Check sheet for the modelled part. Datum: model origin and axes. Units: mm. Face numbers are marked on the shaded views. A direction names the side the tool comes from. Coordinates: 2 decimals unless noted, no trailing zeros. Loops run counter-clockwise (first coordinate to the right, second up) from the corner with the lowest first, then second, coordinate; pieces in that order, holes last.
```python
from build123d import *

# Parameters (mm, degrees)
SKETCH_1_R              = 22.5
EXTRUDE_1_DEPTH         = 705
SKETCH_2_R              = 20.5
EXTRUDE_2_DEPTH         = 39
SKETCH_3_R              = 20
EXTRUDE_3_DEPTH         = 37
SKETCH_4_R              = 19.5
EXTRUDE_4_DEPTH         = 60
SKETCH_5_R              = 17.5
EXTRUDE_5_DEPTH         = 18
EXTRUDE_START           = 39
SKETCH_6_R              = 20.5
EXTRUDE_6_DEPTH         = 39
EXTRUDE_START_2         = 37
SKETCH_7_R              = 20
EXTRUDE_7_DEPTH         = 37
CHAMFER_1_SIZE          = 1
CUT_EXTRUDE_1_DEPTH     = 5.9
CUT_EXTRUDE_2_DEPTH     = 5.73
HOLE_WIZARD_M10_1_D     = 8.5
HOLE_WIZARD_M10_1_DEPTH = 15
HOLE_WIZARD_M10_1_TIP   = 2.553657631


with BuildPart() as part:
    # 草图1 → 凸台-拉伸1 (new body)
    with BuildSketch(Plane(origin=(0, 0, 0), x_dir=(0, 0, -1), z_dir=(1, 0, 0))):
        Circle(SKETCH_1_R)
    extrude(amount=EXTRUDE_1_DEPTH)

    # 草图2 → 凸台-拉伸2 (add)
    with BuildSketch(Plane(origin=(705, 0, 0), x_dir=(0, 0, -1), z_dir=(1, 0, 0))):
        Circle(SKETCH_2_R)
    extrude(amount=EXTRUDE_2_DEPTH)

    # 草图3 → 凸台-拉伸3 (add)
    with BuildSketch(Plane(origin=(744, 0, 0), x_dir=(0, 0, -1), z_dir=(1, 0, 0))):
        Circle(SKETCH_3_R)
    extrude(amount=EXTRUDE_3_DEPTH)

    # 草图4 → 凸台-拉伸4 (add)
    with BuildSketch(Plane(origin=(781, 0, 0), x_dir=(0, 0, -1), z_dir=(1, 0, 0))):
        Circle(SKETCH_4_R)
    extrude(amount=EXTRUDE_4_DEPTH)

    # 草图5 → 凸台-拉伸5 (add)
    with BuildSketch(Plane(origin=(841, 0, 0), x_dir=(0, 0, -1), z_dir=(1, 0, 0))):
        Circle(SKETCH_5_R)
    extrude(amount=EXTRUDE_5_DEPTH)

    # 草图6 → 凸台-拉伸6 (add)
    with BuildSketch(Plane.ZY.offset(EXTRUDE_START)):
        with Locations(Location((0, 0, 0), (0, 0, 180))):
            Circle(SKETCH_6_R)
    extrude(amount=-EXTRUDE_6_DEPTH)

    # 草图7 → 凸台-拉伸7 (add)
    with BuildSketch(Plane.ZY.offset(39).offset(EXTRUDE_START_2)):
        with Locations(Location((0, 0, 0), (0, 0, 180))):
            Circle(SKETCH_7_R)
    extrude(amount=-EXTRUDE_7_DEPTH)

    # 倒角1
    chamfer_1_edges = [part.edges().sort_by_distance(p)[0] for p in [
        (-76, 0, 20),
    ]]
    chamfer(chamfer_1_edges, length=CHAMFER_1_SIZE)

    # 草图8 → 切除-拉伸1 (cut)
    with BuildSketch(Plane(origin=(0, 20.5, 0), x_dir=(1, 0, 0), z_dir=(0, 1, 0))):
        with BuildLine():
            Line((-10, -6), (-30, -6))
            ThreePointArc((-30, -6), (-36, 0), (-30, 6))
            Line((-30, 6), (-10, 6))
            ThreePointArc((-10, 6), (-4, 0), (-10, -6))
        make_face()
        with BuildLine():
            Line((715, 6), (735, 6))
            ThreePointArc((735, 6), (741, 0), (735, -6))
            Line((735, -6), (715, -6))
            ThreePointArc((715, -6), (709, 0), (715, 6))
        make_face()
    extrude(amount=-CUT_EXTRUDE_1_DEPTH, mode=Mode.SUBTRACT)

    # 草图9 → 切除-拉伸2 (cut)
    with BuildSketch(Plane(origin=(0, 17.5, 0), x_dir=(1, 0, 0), z_dir=(0, 1, 0))):
        with BuildLine():
            Line((848, 5), (852, 5))
            ThreePointArc((852, 5), (857, 0), (852, -5))
            Line((852, -5), (848, -5))
            ThreePointArc((848, -5), (843, 0), (848, 5))
        make_face()
    extrude(amount=-CUT_EXTRUDE_2_DEPTH, mode=Mode.SUBTRACT)

    # M10 螺纹孔1
    with Locations(Plane(origin=(859, 0, 0), x_dir=(0, 0, -1), z_dir=(1, 0, 0))):
        with Locations((0, 0)):
            Hole(HOLE_WIZARD_M10_1_D / 2, depth=HOLE_WIZARD_M10_1_DEPTH)
            with Locations((0, 0, -(HOLE_WIZARD_M10_1_DEPTH + HOLE_WIZARD_M10_1_TIP / 2))):  # 118° drill point
                Cone(0, HOLE_WIZARD_M10_1_D / 2, HOLE_WIZARD_M10_1_TIP, mode=Mode.SUBTRACT)


solid = part.part
```
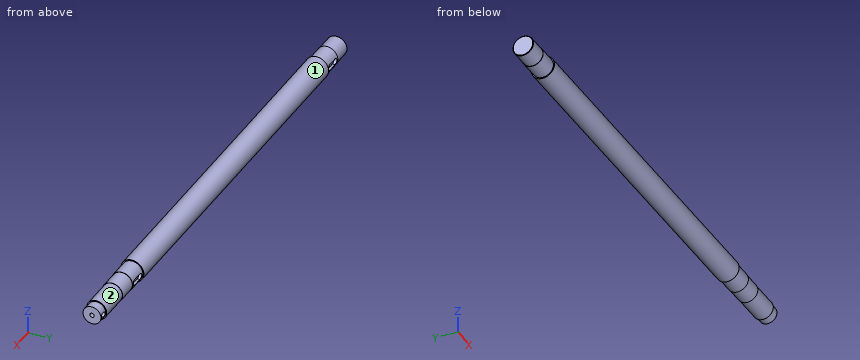
1) Set-up check for the marked faces 1 and 2: record each of +Z, -Z, +X, -X, +Y, -Y from which the full face is reachable in a straight line by a thin tool's end or side.
Answer sheet:
face 1: +X, -X
face 2: +X
2) Section check A-A on x = 168.5. Enter the section's corners in (y, z), plus the area to 3 significant figures.
Answer sheet:
outline: circle Ø45 at (0, 0)
area: 1,590 mm2
3) Depth check by flat-ended pin: pin 1 (1.5 mm diameter, centred on x = 517.5, z = 8.5, fed in from +Y); pin 2 (1.2 mm diameter, centred on x = 849.5, y = 14, fed in from -Z); pin 3 (5 mm diameter, centred on x = 852.5, z = -2.5, fed in from +Y). Enter the tip coordinate at first touch or a pass-through.
Answer sheet:
pin 1: stops at y = 21.12
pin 2: stops at z = -11.26
pin 3: stops at y = 16.85
4) Scan lines: line 1 (Y direction, x = 850.25, z = 0); line 2 (Z direction, x = 382, y = -12); line 3 (Y direction, x = 245.5, z = -2). Record each from-to range of solid material in increasing order.
Answer sheet:
line 1: y = -17.5 to -4.25, 4.25 to 11.77
line 2: z = -19.03 to 19.03
line 3: y = -22.41 to 22.41
